Can you work these out from the model? Positions are in its coordinate system, mm. Round coordinates to 2 decimals unless told otherwise and drop trailing zeros. Write each loop counter-clockwise with the first axis right and the second up, starting at its lowest first coordinate (ties: lowest second). Pieces come first, ordered by that corner, then holes. Notation, with made-up numbers: (43, 40) -> (80, 40) arc R29 ccw to (80, 77) -> close; hole circle Ø4 at (-1, -24). An arc over 180 degrees is marked (long way). Write item = value, one per line. Start each with the question number.
1) If I drill on line 1 (Z direction, x = -15, y = 8.7); line 2 (X direction, y = 8.6, z = 15); line 3 (X direction, y = 8.9, z = -45), over which ranges is the centre line in solid material (lowest first)?
2) Imagine slicing it at C-C, the plane y = 1.5. State how many separate pieces and enclosed holes the cut face has, then the cut area to 3 significant figures.
3) Imagine slicing it at B-B, the plane z = 15. Please give me the cut outline in (x, y).
4) I'm going to push flat-ended pins straight in: pin 1 (6 mm diameter, centred on x = 45, z = -45, fed in from -Y); pin 2 (3.5 mm diameter, centred on x = -44.5, z = 43.5, fed in from -Y); pin 3 (3 mm diameter, centred on y = 9, z = 14.5, fed in from +X). Where does each tip first touch, or does it pass through?
5) Imagine slicing it at A-A, the plane x = 15. Please give me the cut outline in (y, z).
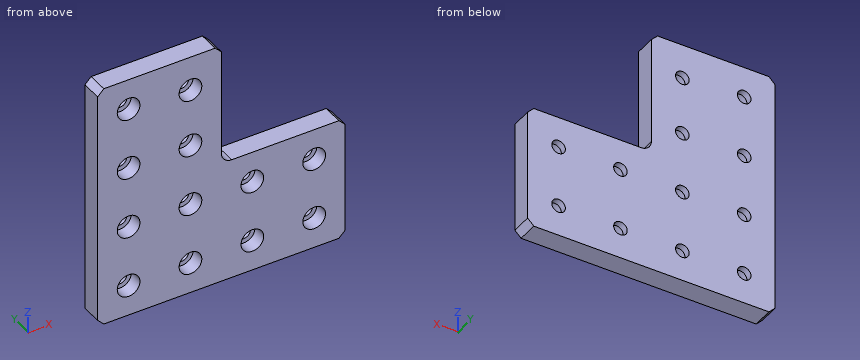
from build123d import *

# Parameters (mm, degrees)
SKETCH_1_W                = 120
SKETCH_1_H                = 120
EXTRUDE_1_DEPTH           = 10
SKETCH_2_W                = 60
SKETCH_2_H                = 60
CUT_EXTRUDE_1_DEPTH       = 25
CHAMFER_1_SIZE            = 3
FILLET_1_R                = 5
HOLE_WIZARD_1_D           = 6.6
HOLE_WIZARD_1_DEPTH       = 25
HOLE_WIZARD_1_CBORE_D     = 11
HOLE_WIZARD_1_CBORE_DEPTH = 6.8
HOLE_WIZARD_1_TIP         = 1.982840043


with BuildPart() as part:
    # 草图1 → 凸台-拉伸1 (new body)
    with BuildSketch(Plane(origin=(0, 0, 0), x_dir=(1, 0, 0), z_dir=(0, 1, 0))):
        Rectangle(SKETCH_1_W, SKETCH_1_H)
    extrude(amount=EXTRUDE_1_DEPTH)

    # 草图2 → 切除-拉伸1 (cut)
    with BuildSketch(Plane(origin=(0, 10, 0), x_dir=(1, 0, 0), z_dir=(0, 1, 0))):
        with Locations((30, -30)):
            Rectangle(SKETCH_2_W, SKETCH_2_H)
    extrude(amount=-CUT_EXTRUDE_1_DEPTH, mode=Mode.SUBTRACT)

    # 倒角1
    chamfer_1_edges = [part.edges().sort_by_distance(p)[0] for p in [
        (60, 5, 0),
        (0, 5, 60),
        (-60, 5, 60),
        (-60, 5, -60),
        (60, 5, -60),
    ]]
    chamfer(chamfer_1_edges, length=CHAMFER_1_SIZE)

    # 圆角1
    fillet_1_edges = [part.edges().sort_by_distance(p)[0] for p in [
        (0, 5, 0),
    ]]
    fillet(fillet_1_edges, radius=FILLET_1_R)

    # 打孔尺寸(%根据)内六角圆柱头螺钉的类型1
    with Locations(Plane(origin=(0, 0, 0), x_dir=(-1, 0, 0), z_dir=(0, -1, 0))):
        with Locations((45, 45), (45, 15), (15, 45), (15, 15), (-45, 45), (-45, 15), (45, -15), (45, -45), (15, -43.223897071), (15, -15), (-15, 45), (-15, 15)):
            CounterBoreHole(HOLE_WIZARD_1_D / 2, HOLE_WIZARD_1_CBORE_D / 2, HOLE_WIZARD_1_CBORE_DEPTH, depth=HOLE_WIZARD_1_DEPTH)
            with Locations((0, 0, -(HOLE_WIZARD_1_DEPTH + HOLE_WIZARD_1_TIP / 2))):  # 118° drill point
                Cone(0, HOLE_WIZARD_1_D / 2, HOLE_WIZARD_1_TIP, mode=Mode.SUBTRACT)


solid = part.part
Reported:
q1.line_1 = -60 to -48.3, -41.7 to -18.3, -11.7 to 11.7, 18.3 to 39.92, 46.52 to 60
q1.line_2 = -60 to -48.3, -41.7 to -18.3, -11.7 to 0
q1.line_3 = -60 to -48.3, -41.7 to -18.3, -11.7 to 11.7, 18.3 to 41.7, 48.3 to 60
q2.separate_pieces = 1
q2.enclosed_holes = 12
q2.area = 9,640 mm²
q3.outline = (-60, 0) -> (-50.5, 0) -> (-50.5, 6.8) -> (-48.3, 6.8) -> (-48.3, 10) -> (-60, 10) -> close; (-41.7, 6.8) -> (-39.5, 6.8) -> (-39.5, 0) -> (-20.5, 0) -> (-20.5, 6.8) -> (-18.3, 6.8) -> (-18.3, 10) -> (-41.7, 10) -> close; (-11.7, 6.8) -> (-9.5, 6.8) -> (-9.5, 0) -> (0, 0) -> (0, 10) -> (-11.7, 10) -> close
q4.pin_1 = through
q4.pin_2 = 6.8
q4.pin_3 = 0
q5.outline = (0, -60) -> (10, -60) -> (10, -48.3) -> (6.8, -48.3) -> (6.8, -50.5) -> (0, -50.5) -> close; (0, -39.5) -> (6.8, -39.5) -> (6.8, -41.7) -> (10, -41.7) -> (10, -18.3) -> (6.8, -18.3) -> (6.8, -20.5) -> (0, -20.5) -> close; (0, -9.5) -> (6.8, -9.5) -> (6.8, -11.7) -> (10, -11.7) -> (10, 0) -> (0, 0) -> close
